Geometry: see drawing. Coordinates: mm, zero at the bounding-box minimum. A direction names the side the tool comes from. Coordinates: 2 decimals unless noted, no trailing zeros. Write each loop counter-clockwise with the first axis right and the second up, starting at its lowest first coordinate (ties: lowest second). Pieces come first, ordered by that corner, then holes. Notation, with made-up numbers: M 17.25,5.5 L 45.25,5.5 A22 cw 45.25,35.5 Z; hole C 82.25,-38 d8. An arc over 180 degrees is marked long. Write item = value, one per line. Start each with the question number.
1. Section query A-A (z = 20.75). Output: boundary loops of the cut face in (x, y), then the cut area to 3 significant figures.
2. Access query for the marked faces 1 and 2. Directions: +Z, -Z, +X, -X, +Y, -Y. A direction counts if a zero-diameter tool reaches every point of the face in a straight line with its end or side. Return the directions, or none.
3. Section query D-D (x = 7.5). Output: boundary loops of the cut face in (y, z).
4. Section query C-C (z = 8). Output: boundary loops of the cut face in (x, y).
5. Section query B-B (y = 7.25). Output: boundary loops of the cut face in (x, z), then the cut area to 3 significant figures.
6. Pin query (flat end, axial travel): pin 1 Ø2 at (y, z) = (1.5, 15.5) entering from +X; pin 2 Ø3 at (y, z) = (3.5, 3) entering from -X; pin 3 Ø4 at (x, z) = (6.5, 10) entering from -Y. Return the tip coordinate at first contact, or that it passes through.
7. Line query: line 1 along Z through (x, y) = (4.5, 6); line 2 along Z through (x, y) = (1.75, 2); line 3 along X through (y, z) = (5.25, 9). Output: solid intervals per line, ascending.
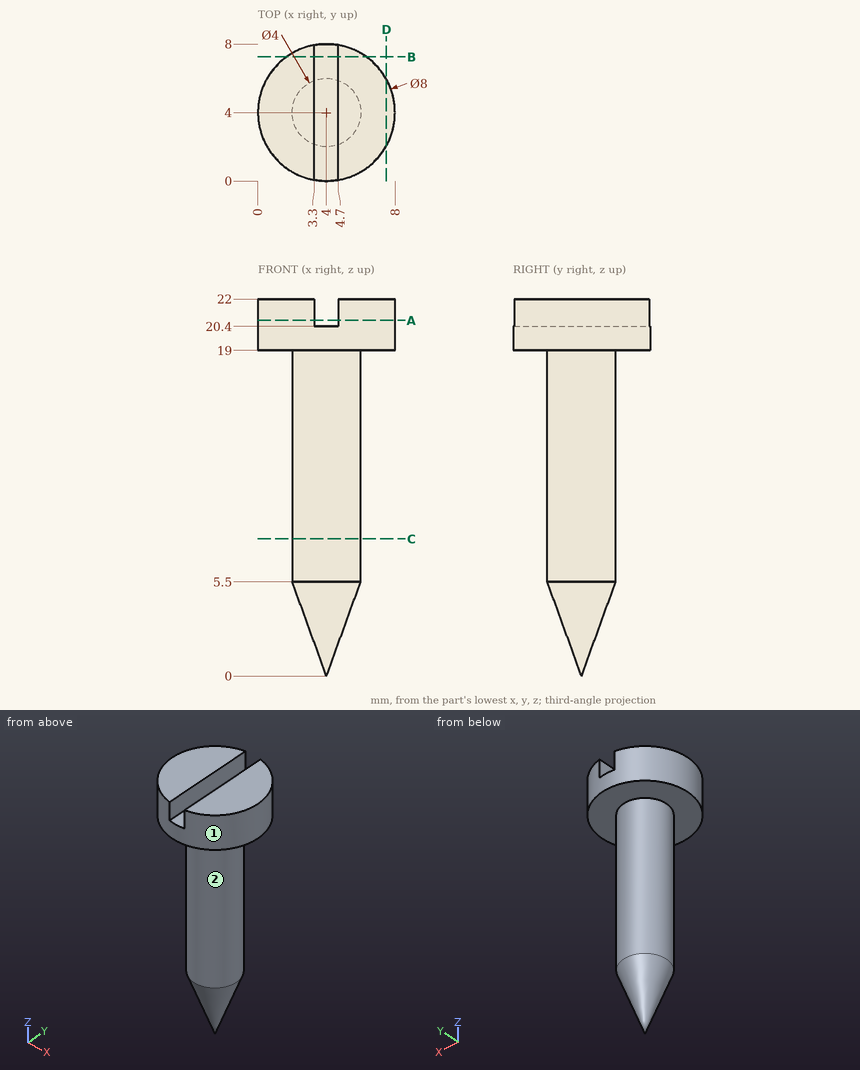
Results are:
q1.outline = M 3.3,0.06 L 3.3,7.94 A4 ccw Z; M 4.7,0.06 A4 ccw 4.7,7.94 Z
q1.area = 39.1 mm^2
q2.face_1 = +Z, -Z
q2.face_2 = -Z
q3.outline = M 2.06,19 L 5.94,19 L 5.94,22 L 2.06,22 Z
q4.outline = C 4,4 d4
q5.outline = M 1.67,19 L 6.33,19 L 6.33,22 L 4.7,22 L 4.7,20.4 L 3.3,20.4 L 3.3,22 L 1.67,22 Z
q5.area = 11.8 mm^2
q6.pin_1 = 5.32
q6.pin_2 = 2.39
q6.pin_3 = 2.06
q7.line_1 = 19 to 20.4
q7.line_2 = 19 to 22
q7.line_3 = 2.44 to 5.56
